Can you work these out from the drawing? Everything is in mm from the part's minimum corner. Give positions to 0.01 mm unless a question says otherwise; leave off trailing zeros. Write each loop counter-clockwise with the first axis right and the second up, starting at its lowest first coordinate (ties: lowest second). Pieces come first, ordered by that corner, then holes. Notation, with made-up numbers: (23, -15) - (28, -15) arc R18 ccw to (28, -4) - close; hole circle Ø3 at (38.5, 22.5). An arc over 180 degrees is marked (long way). Use a Markdown table: item, result.
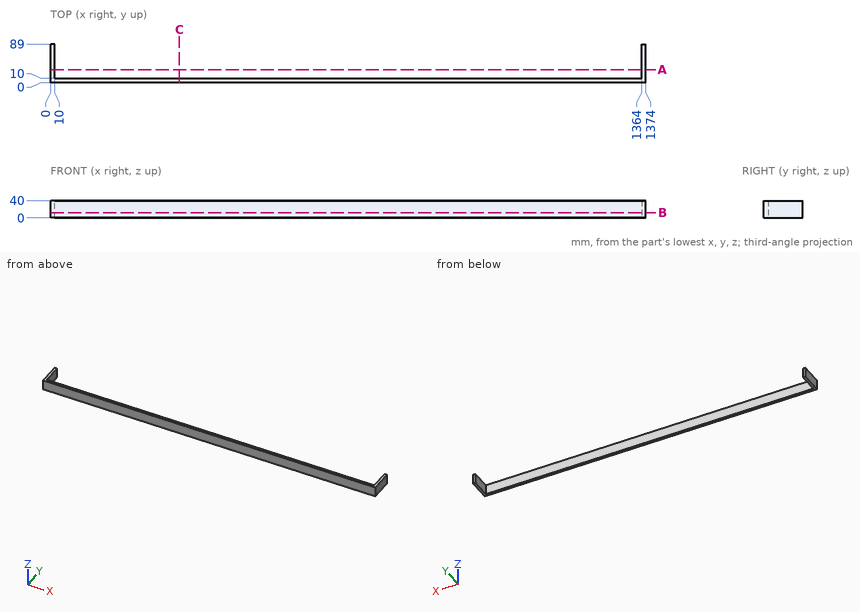
Item 1: If we section it at C-C, the plane x = 297.5: Write out the boundary of the cut face in (y, z), plus the area to 3 significant figures.
Values:
| item | result |
|---|---|
| outline | (0, 0) - (10, 0) - (10, 40) - (0, 40) - close |
| area | 400 mm2 |
Item 2: Will this pin go through, and if not, where does the flat tip stop? pin 1 Ø1.5 at (x, z) = (916.5, 28) entering from +Y.
Values:
| item | result |
|---|---|
| pin 1 | stops at y = 10 |
Item 3: If we section it at B-B, the plane z = 12: Write out the boundary of the cut face in (x, y).
Values:
| item | result |
|---|---|
| outline | (0, 0) - (1374, 0) - (1374, 89) - (1364, 89) - (1364, 10) - (10, 10) - (10, 89) - (0, 89) - close |
Item 4: I need wall thicknesses on line 1 along X through (y, z) = (39.5, 37); line 2 along Y through (x, z) = (63.5, 16.5). Which ranges of each line are inside material? Lowest first, please. Write a range as [from, to].
Values:
| item | result |
|---|---|
| line 1 | x = [0, 10], [1364, 1374] |
| line 2 | y = [0, 10] |
Item 5: If we section it at A-A, the plane y = 30: Write out the boundary of the cut face in (x, z).
Values:
| item | result |
|---|---|
| outline | (0, 0) - (10, 0) - (10, 40) - (0, 40) - close; (1364, 0) - (1374, 0) - (1374, 40) - (1364, 40) - close |
